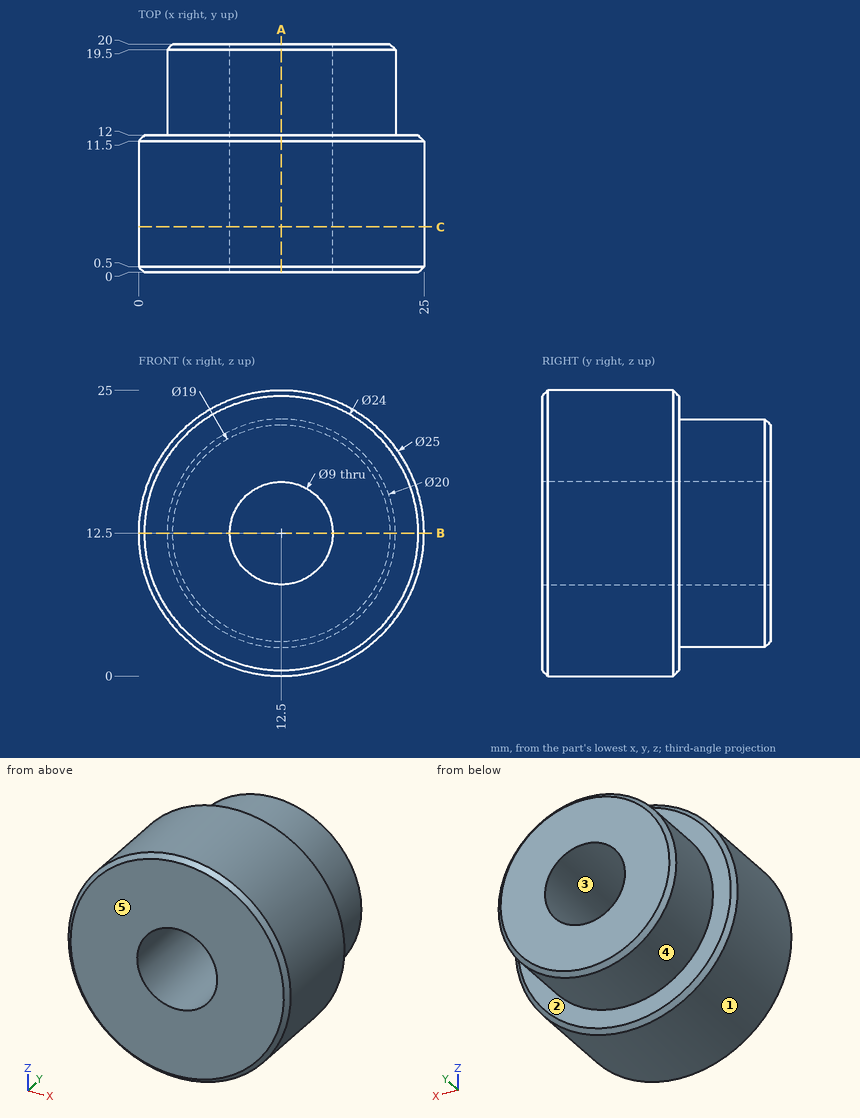
Can you work these out from the drawing? Everything is in mm from the part's minimum corner. A direction names the side the tool comes from. Coordinates: 2 decimals unless noted, no trailing zeros. Loops run counter-clockwise (first coordinate to the right, second up) from the corner with the lowest first, then second, coordinate; pieces in that order, holes last.
1. Imagine slicing it at B-B, the plane z = 12.5. Please give me the cut outline in (x, y).
2. For the marked faces 4 and 5, which set-ups out of +Z, -Z, +X, -X, +Y, -Y let a thin tool reach every point of the face, with its end or its side?
3. If we mould it in two halves opening along X, with no side actions, what happens to the marked faces 1, 2 and 3? For each: pulls with the +X half, pulls with the -X half, needs draft (parallel to the pull), parting line crosses it, or undercut.
4. Imagine slicing it at A-A, the plane x = 12.5. Please give me the cut outline in (y, z), and give its area (3 significant figures).
5. I need wall thicknesses on L1, parallel to X at y = 7, z = 12.5; L2, parallel to X at y = 15.25, z = 12.5; L3, parallel to Y at x = 4.25, z = 19.5. Which ranges of each line are inside material? Lowest first, please.
6. For P1, Ø8, axis at y = 12.5, z = 10.5, coming from the +X side; P2, Ø1.5, axis at x = 11.5, y = 13, coming from the -Z side; P3, Ø5, axis at y = 3.5, z = 7.5, coming from the +X side, each with a flat end and sliding along its axis, tell me the tip position at first contact or that it passes through.
7. Imagine slicing it at C-C, the plane y = 4. Please give me the cut outline in (x, z).
Taken from the geometry:
1. outline: (0, 0.5) - (0.5, 0) - (8, 0) - (8, 20) - (3, 20) - (2.5, 19.5) - (2.5, 12) - (0.5, 12) - (0, 11.5) - close; (17, 0) - (24.5, 0) - (25, 0.5) - (25, 11.5) - (24.5, 12) - (22.5, 12) - (22.5, 19.5) - (22, 20) - (17, 20) - close
2. face 4: +Y
2. face 5: +Z, -Z, +X, -X, -Y
3. face 1: parting line crosses it
3. face 2: needs draft
3. face 3: undercut
4. outline: (0, 0.5) - (0.5, 0) - (11.5, 0) - (12, 0.5) - (12, 2.5) - (19.5, 2.5) - (20, 3) - (20, 8) - (0, 8) - close; (0, 17) - (20, 17) - (20, 22) - (19.5, 22.5) - (12, 22.5) - (12, 24.5) - (11.5, 25) - (0.5, 25) - (0, 24.5) - close
4. area: 279 mm2
5. L1: x = 0 to 8, 17 to 25
5. L2: x = 2.5 to 8, 17 to 22.5
5. L3: y = 0 to 12
6. P1: stops at x = 25
6. P2: stops at z = 2.5
6. P3: stops at x = 24.75
7. outline: circle Ø25 at (12.5, 12.5); hole circle Ø9 at (12.5, 12.5)
